from build123d import *

# Parameters (mm, degrees)
BOSS_EXTRUDE1_DEPTH = 4


with BuildPart() as part:
    # Sketch1 → Boss-Extrude1 (new, symmetric)
    with BuildSketch(Plane.XY):
        with BuildLine():
            Line((-31.75, 73.26818434), (-31.75, -73.26818434))
            ThreePointArc((-31.75, -73.26818434), (-27.614383176, -83.610581461), (-17.487976239, -88.250019711))
            Line((-17.487976239, -88.250019711), (31.75, -90.675387205))
            Line((31.75, -90.675387205), (31.75, 90.675387205))
            Line((31.75, 90.675387205), (-17.487976239, 88.250019711))
            ThreePointArc((-17.487976239, 88.250019711), (-27.614383176, 83.610581461), (-31.75, 73.26818434))
        make_face()
    extrude(amount=BOSS_EXTRUDE1_DEPTH, both=True)


solid = part.part
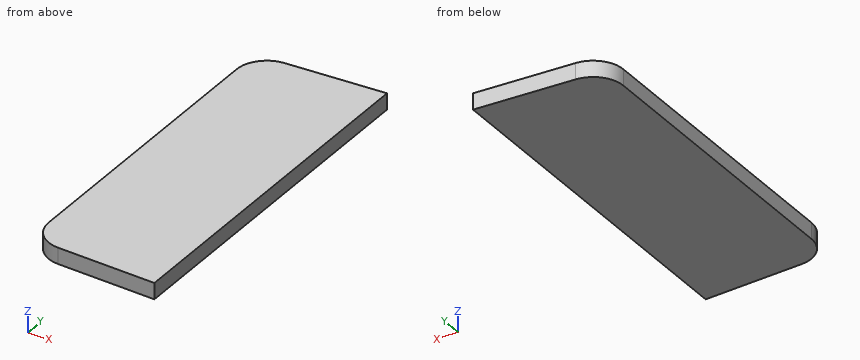
Could you check a few things on this model? Use its own coordinates, in mm. Give positions to 0.01 mm unless a question says otherwise; leave off trailing zeros. Order: outer loops, then holes, each group sorted by start corner. A loop starts at its lowest first (then second) coordinate and runs counter-clockwise, first axis right, second up.
1. Suppose I cut it at B-B (x = -12). Write out the boundary of the cut face in (y, z), plus the area to 3 significant figures.
Answers below:
outline: (-88.52, -4) - (88.52, -4) - (88.52, 4) - (-88.52, 4) - close
area: 1,420 mm2
2. For pin 1 (1.5 mm diameter, centred on x = -22, z = -2.5, fed in from -Y); pin 2 (4 mm diameter, centred on x = 0, z = -1, fed in from -Y); pin 3 (1 mm diameter, centred on x = 15.5, z = -2.5, fed in from -Y), each with a flat end and sliding along its axis, tell me the tip position at first contact or that it passes through.
Answers below:
pin 1: stops at y = -87.58
pin 2: stops at y = -89.21
pin 3: stops at y = -89.9
3. Suppose I cut it at C-C (x = -22.5). Write out the boundary of the cut face in (y, z), plus the area to 3 significant figures.
Answers below:
outline: (-87.12, -4) - (87.12, -4) - (87.12, 4) - (-87.12, 4) - close
area: 1,390 mm2
4. I need wall thicknesses on L1, parallel to Y at x = 25, z = -1; L2, parallel to X at y = 79, z = 1.5; L3, parallel to X at y = 81, z = -1.5. Which ranges of each line are inside material? Lowest first, please.
Answers below:
L1: y = -90.34 to 90.34
L2: x = -30.61 to 31.75
L3: x = -29.6 to 31.75
5. Suppose I cut it at A-A (z = 1.5). Write out the boundary of the cut face in (x, y), plus the area to 3 significant figures.
Answers below:
outline: (-31.75, -73.27) arc R15 ccw to (-17.49, -88.25) - (31.75, -90.68) - (31.75, 90.68) - (-17.49, 88.25) arc R15 ccw to (-31.75, 73.27) - close
area: 11,200 mm2
